from build123d import *

# Parameters (mm, degrees)
SKETCH_1_R           = 2.8
BOSS_EXTRUDE_1_DEPTH = 1.8
SKETCH_4_R           = 1.375
BOSS_EXTRUDE_2_DEPTH = 0.7
SKETCH_6_R           = 1.425
BOSS_EXTRUDE_3_DEPTH = 3
SKETCH_8_W           = 1.368195424
SKETCH_8_H           = 0.8
CUT_EXTRUDE_1_DEPTH  = 8.429670248


with BuildPart() as part:
    # Sketch 1 → Boss-Extrude 1 (new body)
    with BuildSketch(Plane.XY):
        Circle(SKETCH_1_R)
    extrude(amount=BOSS_EXTRUDE_1_DEPTH)

    # Sketch 3 → Revolve 1 (revolve)
    with BuildSketch(Plane(origin=(0, 0, 0), x_dir=(1, 0, 0), z_dir=(0, 1, 0))):
        with BuildLine():
            Line((0, 0), (1.475, 0))
            ThreePointArc((1.475, 0), (1.42299689, 0.04799689), (1.375, 0.1))
            Line((1.375, 0.1), (0, 0.1))
            Line((0, 0.1), (0, 0))
        make_face()
    revolve(axis=Axis((0, 0, 0), (0, 0, -1)))

    # Sketch 4 → Boss-Extrude 2 (add)
    with BuildSketch(Plane(origin=(0, 0, -0.1), x_dir=(-1, 0, 0), z_dir=(0, 0, -1))):
        Circle(SKETCH_4_R)
    extrude(amount=BOSS_EXTRUDE_2_DEPTH)

    # Sketch 5 → Revolve 2 (revolve)
    with BuildSketch(Plane(origin=(0, 0, 0), x_dir=(1, 0, 0), z_dir=(0, 1, 0)), mode=Mode.PRIVATE) as revolve_2_sk:
        Polygon((0, 0.8), (1.375, 0.8), (1.425, 1), (0, 1), align=None)
    revolve(revolve_2_sk.sketch.rotate(Axis((0, 0, 0), (0, 0, -1)), 180), axis=Axis((0, 0, 0), (0, 0, -1)))

    # Sketch 6 → Boss-Extrude 3 (add)
    with BuildSketch(Plane(origin=(0, 0, -1), x_dir=(-1, 0, 0), z_dir=(0, 0, -1))):
        Circle(SKETCH_6_R)
    extrude(amount=BOSS_EXTRUDE_3_DEPTH)

    # Sketch 7 → Cut-Revolve 3 (revolve, cut)
    with BuildSketch(Plane(origin=(0, 0, 0), x_dir=(1, 0, 0), z_dir=(0, 1, 0)), mode=Mode.PRIVATE) as cut_revolve_3_sk:
        with BuildLine():
            Line((1.82, -1.8), (2.8, -1.8))
            Line((2.8, -1.8), (2.8, -0.98))
            ThreePointArc((2.8, -0.98), (2.429916567, -1.533314921), (1.82, -1.8))
        make_face()
    revolve(cut_revolve_3_sk.sketch.rotate(Axis((0, 0, -0.11680497), (0, 0, 1)), 180), axis=Axis((0, 0, -0.11680497), (0, 0, 1)), mode=Mode.SUBTRACT)

    # Sketch 8 → Cut-Extrude 1 (cut, through all)
    with BuildSketch(Plane.ZY.offset(2.8)):
        with Locations((1.384097712, 0)):
            Rectangle(SKETCH_8_W, SKETCH_8_H)
    extrude(amount=-CUT_EXTRUDE_1_DEPTH, mode=Mode.SUBTRACT)


solid = part.part
Verification items for the finished model (mm, model axes). A direction names the side the tool comes from. Coordinates: 2 decimals unless noted, no trailing zeros. Order: outer loops, then holes, each group sorted by start corner. A loop starts at its lowest first (then second) coordinate and runs counter-clockwise, first axis right, second up. Notation, with made-up numbers: (22.5, 27) -> (27.5, 27) arc R24 ccw to (27.5, 65) -> close; hole circle Ø6 at (-32, 35.25). An arc over 180 degrees is marked (long way). Put each result on its own line as item: value. Start each with the question number.
1. Go/stop test with flat-tipped pins: pin 1 Ø1.7 at (x, y) = (0.5, 1.5) entering from -Z; pin 2 Ø0.9 at (x, z) = (-1, 1) entering from -Y; pin 3 Ø2 at (x, z) = (1.5, 1) entering from -Y. Record where each tip stops, or that it passes through.
2. Cross-section at D-D, the plane z = -0.7. Record the boundary of the cut face in (x, y) (3 decimals).
3. Access from +Z, -Z, +X, -X, +Y, -Y to the whole of each face (thin tool, end or side, straight path). Record for faces 4 (the flat face through (0, 0.4, 1)), 5 (the flat face through (0, -1, 1.8)), 6 (the flat face through (1.2, -1.2, 0)), 7 (the cylindrical face through (0.3, -1.34, -0.45)).
4. Cross-section at B-B, the plane x = 0. Record the boundary of the cut face in (y, z) (3 decimals), then the cut area to 3 significant figures.
5. Cross-section at C-C, the plane z = -1.45. Record the boundary of the cut face in (x, y) (3 decimals).
6. Cross-section at A-A, the plane y = 0. Record the boundary of the cut face in (x, z) (3 decimals), then the cut area to 3 significant figures.
7. Mould release check, pull along Y, two halves, no side actions. Record for faces 1 (the flat face through (0, 0, 0.7)), 2 (the flat face through (0, 1, 1.8)), 3 (the cylindrical face through (1.13, -0.87, -2.48)): released by +Y, released by -Y, zero draft, split by the parting line, or undercut.
8. Material ranges on L1, parallel to Y at x = -0.05, z = 0.9; L2, parallel to Y at x = 1.75, z = 1; L3, parallel to Z at x = 0.9, y = 0, recorded low to high. Write a range as [from, to].
Computed:
1. pin 1: z = -4
1. pin 2: y = -2.75
1. pin 3: y = -2.75
2. outline: circle Ø2.75 at (0, 0)
3. face 4: +Z, +X, -X
3. face 5: +Z, +X, -X, +Y, -Y
3. face 6: -Z
3. face 7: none
4. outline: (-2.8, 0) -> (-1.475, 0) arc R0.884 cw to (-1.375, -0.1) -> (-1.375, -0.8) -> (-1.425, -1) -> (-1.425, -4) -> (1.425, -4) -> (1.425, -1) -> (1.375, -0.8) -> (1.375, -0.1) arc R0.884 cw to (1.475, 0) -> (2.8, 0) -> (2.8, 0.98) arc R1.186 ccw to (1.82, 1.8) -> (0.4, 1.8) -> (0.4, 0.7) -> (-0.4, 0.7) -> (-0.4, 1.8) -> (-1.82, 1.8) arc R1.186 ccw to (-2.8, 0.98) -> close
4. area: 20.0 mm2
5. outline: circle Ø2.85 at (0, 0)
6. outline: (-2.8, 0) -> (-1.475, 0) arc R0.884 cw to (-1.375, -0.1) -> (-1.375, -0.8) -> (-1.425, -1) -> (-1.425, -4) -> (1.425, -4) -> (1.425, -1) -> (1.375, -0.8) -> (1.375, -0.1) arc R0.884 cw to (1.475, 0) -> (2.8, 0) -> (2.8, 0.7) -> (-2.8, 0.7) -> close
6. area: 15.2 mm2
7. face 1: undercut
7. face 2: zero draft
7. face 3: split by the parting line
8. L1: [-2.8, -0.4], [0.4, 2.8]
8. L2: [-2.18, -0.4], [0.4, 2.18]
8. L3: [-4, 0.7]
